Geometry: final body of the model. Coordinates: model frame, mm. Coordinates: 2 decimals unless noted, no trailing zeros. Write each loop counter-clockwise with the first axis right and the second up, starting at its lowest first coordinate (ties: lowest second). Pieces come first, ordered by that corner, then holes. Notation, with made-up numbers: (-1.5, 52.25) -> (3.5, 52.25) arc R33 ccw to (3.5, 86.25) -> close; hole circle Ø3 at (-15.75, 59.5). An arc over 180 degrees is marked (long way). Answer as a JSON object with one key per item and string values. Group by question number.
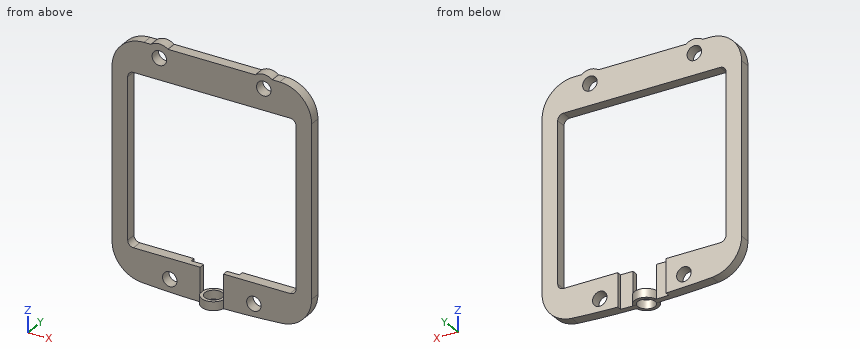
```python
from build123d import *
from build123d.topology import SkipClean

# Parameters (mm, degrees)
BOSS_EXTRUDE_1_DEPTH      = 0.9
CUT_EXTRUDE_1_DEPTH       = 28.026205
CUT_EXTRUDE_1_DEPTH_BACK  = 28.026205
SKETCH_2_R                = 1.25
SKETCH_3_W                = 4
SKETCH_3_H                = 4.342956
CUT_EXTRUDE_2_DEPTH       = 1.8
SKETCH_4_W                = 8.3
SKETCH_4_H                = 6.175349
CUT_EXTRUDE3_DEPTH        = 0.8
BOSS_EXTRUDE_2_REACH      = 45.477
BOSS_EXTRUDE_2_END_RADIUS = 173.987356
SKETCH_10_R               = 2.061553
SKETCH_10_R_2             = 1.5
SKETCH_11_R               = 1.5
CUT_EXTRUDE_7_DEPTH       = 10


with BuildPart() as part:
    # Sketch 1 → Boss-Extrude 1 (new, symmetric)
    with BuildSketch(Plane(origin=(0, 0, 0), x_dir=(1, 0, 0), z_dir=(0, 1, 0))):
        with BuildLine():
            Line((-17.2, -14.827044), (-17.2, 14.686233))
            ThreePointArc((-17.2, 14.686233), (-15.721853, 18.437859), (-12.081928, 20.172956))
            ThreePointArc((-12.081928, 20.172956), (0, 20.592956), (12.081928, 20.172956))
            ThreePointArc((12.081928, 20.172956), (15.721853, 18.437859), (17.2, 14.686233))
            Line((17.2, 14.686233), (17.2, -14.827044))
            ThreePointArc((17.2, -14.827044), (15.589087, -18.716131), (11.7, -20.327044))
            Line((11.7, -20.327044), (10.41998, -20.327044))
            ThreePointArc((10.41998, -20.327044), (8.953692, -20.827044), (7.487405, -20.327044))
            Line((7.487405, -20.327044), (-7.583712, -20.327044))
            ThreePointArc((-7.583712, -20.327044), (-9.05, -20.827044), (-10.516288, -20.327044))
            Line((-10.516288, -20.327044), (-11.7, -20.327044))
            ThreePointArc((-11.7, -20.327044), (-15.589087, -18.716131), (-17.2, -14.827044))
        make_face()
        with BuildLine():
            Line((-13.5, -14.75), (13.5, -14.75))
            ThreePointArc((13.5, -14.75), (14.207107, -14.457107), (14.5, -13.75))
            Line((14.5, -13.75), (14.5, 13.75))
            ThreePointArc((14.5, 13.75), (14.207107, 14.457107), (13.5, 14.75))
            Line((13.5, 14.75), (-13.5, 14.75))
            ThreePointArc((-13.5, 14.75), (-14.207107, 14.457107), (-14.5, 13.75))
            Line((-14.5, 13.75), (-14.5, -13.75))
            ThreePointArc((-14.5, -13.75), (-14.207107, -14.457107), (-13.5, -14.75))
        make_face(mode=Mode.SUBTRACT)
    extrude(amount=BOSS_EXTRUDE_1_DEPTH, both=True)

    # Sketch 2 → Cut-Extrude 1 (cut, two sides: drawn at the far end of the back side and taken through both)
    with BuildSketch(Plane(origin=(0, 0, 0), x_dir=(1, 0, 0), z_dir=(0, 1, 0)).offset(-CUT_EXTRUDE_1_DEPTH_BACK)):
        with Locations(Location((-9.05, -18.427044, 0), (0, 0, 270))):
            Circle(SKETCH_2_R)
        with Locations(Location((8.953692, -18.427044, 0), (0, 0, 270))):
            Circle(SKETCH_2_R)
        with Locations(Location((-7.253142, 18.256885, 0), (0, 0, 270))):
            Circle(SKETCH_2_R)
        with Locations(Location((7.253142, 18.256885, 0), (0, 0, 270))):
            Circle(SKETCH_2_R)
    extrude(amount=CUT_EXTRUDE_1_DEPTH + CUT_EXTRUDE_1_DEPTH_BACK, mode=Mode.SUBTRACT)

    # Sketch 3 → Cut-Extrude 2 (cut)
    with BuildSketch(Plane(origin=(0, 0.9, 0), x_dir=(1, 0, 0), z_dir=(0, 1, 0))):
        with Locations((0, 16.921478)):
            Rectangle(SKETCH_3_W, SKETCH_3_H)
    extrude(amount=-CUT_EXTRUDE_2_DEPTH, mode=Mode.SUBTRACT)

    # Sketch 4 → Cut-Extrude3 (cut)
    with BuildSketch(Plane(origin=(0, 0.9, 0), x_dir=(1, 0, 0), z_dir=(0, 1, 0))):
        with Locations((0, 17.837674)):
            Rectangle(SKETCH_4_W, SKETCH_4_H)
    extrude(amount=-CUT_EXTRUDE3_DEPTH, mode=Mode.SUBTRACT)

    # Boss-Extrude 2: up to this cylinder (the profile starts inside it)
    boss_extrude_2_end = Plane(origin=(0, -0.4, 153.3944), z_dir=(0, -1, 0)) * Cylinder(BOSS_EXTRUDE_2_END_RADIUS, 439.928711, mode=Mode.PRIVATE)
    # Sketch 10 → Boss-Extrude 2 (add, up to the surface)
    with BuildSketch(Plane.XY.offset(-19.092956), mode=Mode.PRIVATE) as boss_extrude_2_sk1:
        with Locations((0, -0.4)):
            Circle(SKETCH_10_R)
        with Locations((0, -0.4)):
            Circle(SKETCH_10_R_2, mode=Mode.SUBTRACT)
    boss_extrude_2_tool1 = extrude(boss_extrude_2_sk1.sketch, amount=-BOSS_EXTRUDE_2_REACH, mode=Mode.PRIVATE) & boss_extrude_2_end
    add(boss_extrude_2_tool1.solids().sort_by_distance((-2.003243, -0.4, -19.092956))[0])

    # Sketch 11 → Cut-Extrude 7 (cut)
    with SkipClean():  # the faces are left unmerged after this step: merging them gives an invalid solid
        with BuildSketch(Plane.XY.offset(-19.092956)):
            with Locations((0, -0.4)):
                Circle(SKETCH_11_R)
        extrude(amount=-CUT_EXTRUDE_7_DEPTH, mode=Mode.SUBTRACT)


solid = part.part
```
Item 1: Section A-A on z = 3. Output: boundary loops of the cut face in (x, y), then the cut area to 3 significant figures.
Item 2: Ray query, L1, parallel to X at y = -0.1, z = 4.5; L2, parallel to Z at x = -9.05, y = 0.1; L3, parallel to Y at x = 0, z = -20.1. Return the intervals inside material, ascending. Write a range as [from, to].
Item 3: Section D-D on x = -9.05. Output: boundary loops of the cut face in (y, z), then the cut area to 3 significant figures.
Item 4: Contact query for flat-ended pins moving along their axis: pin 1 (0.9 mm diameter, centred on y = 0.5, z = -18, fed in from +X); pin 2 (1.1 mm diameter, centred on x = 3, z = -16.5, fed in from +Y); pin 3 (0.5 mm diameter, centred on x = 7.5, y = 0.5, fed in from +Z). Output: stop coordinate, or through.
Item 5: Section B-B on x = 6.5. Output: boundary loops of the cut face in (y, z).
Item 6: Section C-C on y = -1.4. Output: boundary loops of the cut face in (x, z), then the cut area to 3 significant figures.
Answer sheet:
{
 "1": {"outline": "(-17.2, -0.9) -> (-14.5, -0.9) -> (-14.5, 0.9) -> (-17.2, 0.9) -> close; (14.5, -0.9) -> (17.2, -0.9) -> (17.2, 0.9) -> (14.5, 0.9) -> close", "area": "9.72 mm^2"},
 "2": {"L1": "x = [-17.2, -14.5], [14.5, 17.2]", "L2": "z = [-20.36, -14.75], [14.75, 17.18], [19.68, 20.83]", "L3": "y = [-2.46, -1.9], [1.1, 1.66]"},
 "3": {"outline": "(-0.9, -20.36) -> (0.9, -20.36) -> (0.9, -14.75) -> (-0.9, -14.75) -> close; (-0.9, 14.75) -> (0.9, 14.75) -> (0.9, 17.18) -> (-0.9, 17.18) -> close; (-0.9, 19.68) -> (0.9, 19.68) -> (0.9, 20.83) -> (-0.9, 20.83) -> close", "area": "16.5 mm^2"},
 "4": {"pin 1": "stops at x = 16.4", "pin 2": "stops at y = 0.1", "pin 3": "stops at z = 20.5"},
 "5": {"outline": "(-0.9, -20.47) -> (0.9, -20.47) -> (0.9, -19.25) -> (-0.9, -19.25) -> close; (-0.9, -17.26) -> (0.9, -17.26) -> (0.9, -14.75) -> (-0.9, -14.75) -> close; (-0.9, 14.75) -> (0.9, 14.75) -> (0.9, 20.33) -> (-0.9, 20.33) -> close"},
 "6": {"outline": "(-1.8, -20.58) arc R173.99 ccw to (-1.12, -20.59) -> (-1.12, -19.09) -> (-1.8, -19.09) -> close; (1.12, -20.59) arc R173.99 ccw to (1.8, -20.58) -> (1.8, -19.09) -> (1.12, -19.09) -> close", "area": "2.05 mm^2"}
}
